Source: three-view drawing plus pictorial views. Frame: mm from the lowest corner of the part. Give positions to 0.01 mm unless a question says otherwise; leave off trailing zeros. Order: outer loops, then holes, each group sorted by start corner. A loop starts at its lowest first (then second) coordinate and runs counter-clockwise, first axis right, second up. Notation, with made-up numbers: (-13.5, 20.5) -> (44.5, 20.5) arc R31 ccw to (44.5, 58.5) -> close; hole circle Ø9 at (34, -24). An arc over 180 degrees is marked (long way). Answer in a Markdown table with one row per item. Add a question column.
Q1. Cut plane B-B on z = 2. Return the cut outline in (x, y).
Q2. Cut plane D-D on y = 220. Return the cut outline in (x, z), and give its area (3 significant figures).
Q3. Cut plane A-A on x = 20. Count the separate pieces of the cut face and the enclosed holes in it, and give its area (4 significant figures).
Q4. Cut plane C-C on y = 35. Return the cut outline in (x, z).
Q5. Line query: line 1 along X through (y, z) = (37, 1.6); line 2 along X through (y, z) = (225, 2.6); line 3 along Y through (x, z) = (26.5, 2.75). Output: solid intervals per line, ascending. Write a range as from..to.
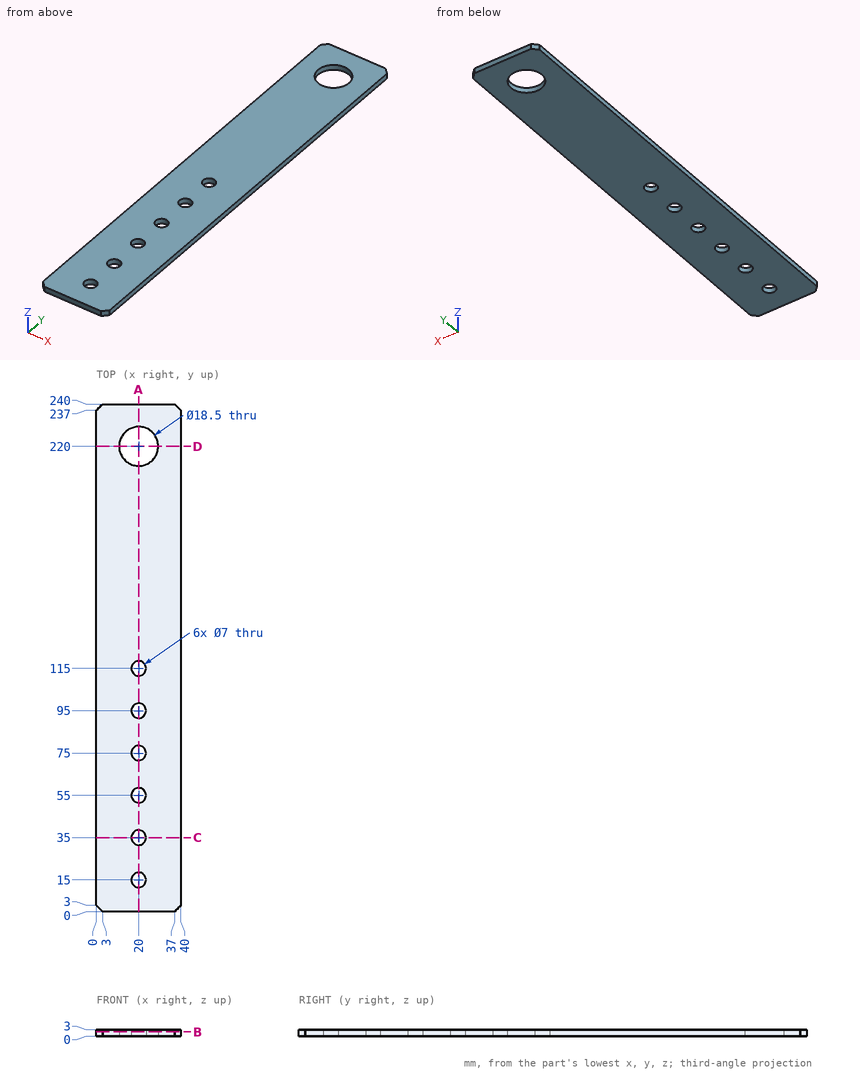
Completed:
| question | item | result |
|---|---|---|
| 1 | outline | (0, 3) -> (3, 0) -> (37, 0) -> (40, 3) -> (40, 237) -> (37, 240) -> (3, 240) -> (0, 237) -> close; hole circle Ø18.5 at (20, 220); hole circle Ø7 at (20, 15); hole circle Ø7 at (20, 35); hole circle Ø7 at (20, 55); hole circle Ø7 at (20, 75); hole circle Ø7 at (20, 95); hole circle Ø7 at (20, 115) |
| 2 | outline | (0, 0) -> (10.75, 0) -> (10.75, 3) -> (0, 3) -> close; (29.25, 0) -> (40, 0) -> (40, 3) -> (29.25, 3) -> close |
| 2 | area | 64.5 mm² |
| 3 | separate pieces | 8 |
| 3 | enclosed holes | 0 |
| 3 | area | 538.5 mm² |
| 4 | outline | (0, 0) -> (16.5, 0) -> (16.5, 3) -> (0, 3) -> close; (23.5, 0) -> (40, 0) -> (40, 3) -> (23.5, 3) -> close |
| 5 | line 1 | x = 0..17.13, 22.87..40 |
| 5 | line 2 | x = 0..12.22, 27.78..40 |
| 5 | line 3 | y = 0..213.42, 226.58..240 |
